The figure shows three views and two pictorial views of one solid part (mm, origin at its lowest corner). Answer the questions. Give positions to 0.01 mm unless a question says otherwise; leave off trailing zeros. Loops run counter-clockwise (first coordinate to the right, second up) from the corner with the lowest first, then second, coordinate; pieces in that order, holes last. Notation, with made-up numbers: (-40, 32) - (13, 32) arc R22 cw to (13, 40) - close; hole circle Ø11 at (16.5, 62.25). An arc over 180 degrees is marked (long way). Use a Markdown table: item, result. Add a question column.
Item 1: Consider probe 1 along Y at (x, z) = (128.5, 4.5); probe 2 along Y at (x, z) = (207, 7.75); probe 3 along Y at (x, z) = (15, 10.25). Determine where each line is inside the solid, lowest interval first. Write a range as [from, to].
Item 2: A cutting plane is placed at A-A (x = 130). Determine the outline of the cut face in (y, z), plus the area to 4 significant figures.
Item 3: A cutting plane is placed at C-C (x = 245). Determine the outline of the cut face in (y, z).
Item 4: Each of these flat-tipped pins is pushed along its axis until it touches: P1, Ø2, axis at y = 172.5, z = 11.5, coming from the +X side; P2, Ø3, axis at y = 29.5, z = 11.5, coming from the +X side (1 decimal); P3, Ø8, axis at x = 29, z = 6.5, coming from the -Y side. Where does it stop, or does it pass through?
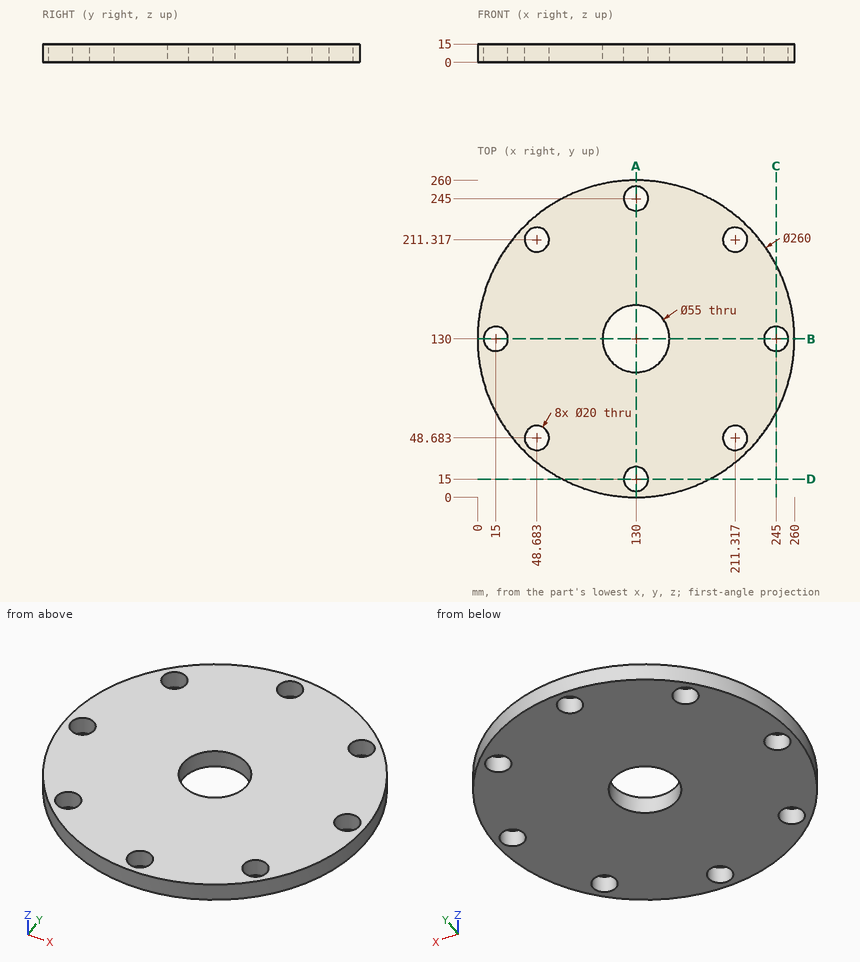
Geometry says:
| question | item | result |
|---|---|---|
| 1 | probe 1 | [0.01, 5.11], [24.89, 102.54], [157.46, 235.11], [254.89, 259.99] |
| 1 | probe 2 | [25.26, 39.66], [57.7, 202.3], [220.34, 234.74] |
| 1 | probe 3 | [69.38, 120], [140, 190.62] |
| 2 | outline | (0, 0) - (5, 0) - (5, 15) - (0, 15) - close; (25, 0) - (102.5, 0) - (102.5, 15) - (25, 15) - close; (157.5, 0) - (235, 0) - (235, 15) - (157.5, 15) - close; (255, 0) - (260, 0) - (260, 15) - (255, 15) - close |
| 2 | area | 2,475 mm² |
| 3 | outline | (69.38, 0) - (120, 0) - (120, 15) - (69.38, 15) - close; (140, 0) - (190.62, 0) - (190.62, 15) - (140, 15) - close |
| 4 | P1 | x = 253.2 |
| 4 | P2 | x = 214.3 |
| 4 | P3 | y = 43.45 |
